Geometry: see drawing. Coordinates: mm, zero at the bounding-box minimum. Round coordinates to 2 decimals unless told otherwise and drop trailing zeros. Write each loop counter-clockwise with the first axis right and the second up, starting at its lowest first coordinate (ties: lowest second). Pieces come first, ordered by that corner, then holes. Notation, with made-up numbers: M 7.5,-30 L 27.5,-30 A30 cw 27.5,-5 Z; hole C 72,-28 d3. An arc over 180 degrees is marked long. Write each question's results on one line, items separated by ' | '. Start each with the question number.
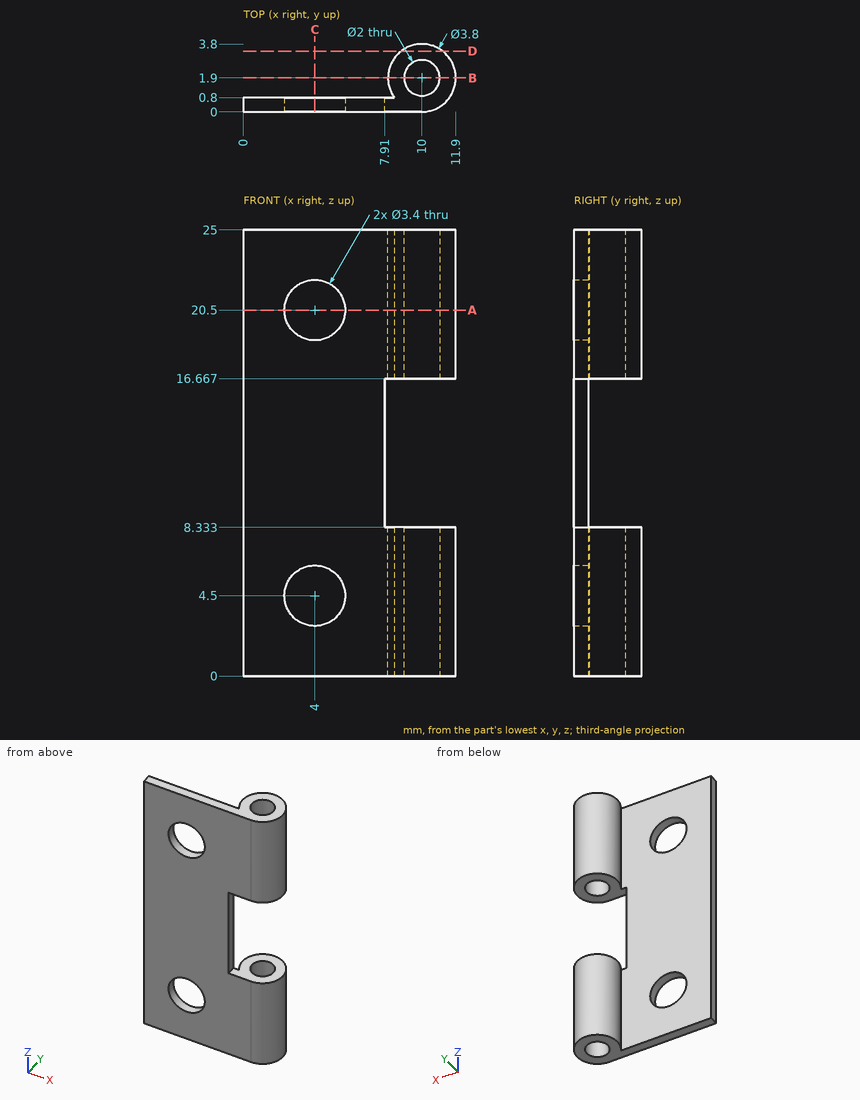
1. Cut plane D-D on y = 3.4. Output: boundary loops of the cut face in (x, z).
2. Cut plane B-B on y = 1.9. Output: boundary loops of the cut face in (x, z).
3. Cut plane A-A on z = 20.5. Output: boundary loops of the cut face in (x, y), and give its area (3 significant figures).
4. Contact query for a flat-ended pin moving along its axis: P1, Ø1.1, axis at x = 9.5, y = 1.5, coming from the -Z side. Output: stop coordinate, or through.
5. Cut plane C-C on x = 4. Output: boundary loops of the cut face in (y, z).
6. Line query: L1, parallel to X at y = 1.85, z = 3.5; L2, parallel to Z at x = 9.75, y = 3.15; L3, parallel to Y at x = 5.25, z = 16. Output: solid intervals per line, ascending. Write a range as from..to.
Answers follow:
1) outline: M 8.83,0 L 11.17,0 L 11.17,8.33 L 8.83,8.33 Z; M 8.83,16.67 L 11.17,16.67 L 11.17,25 L 8.83,25 Z
2) outline: M 8.1,0 L 9,0 L 9,8.33 L 8.1,8.33 Z; M 8.1,16.67 L 9,16.67 L 9,25 L 8.1,25 Z; M 11,0 L 11.9,0 L 11.9,8.33 L 11,8.33 Z; M 11,16.67 L 11.9,16.67 L 11.9,25 L 11,25 Z
3) outline: M 0,0 L 2.3,0 L 2.3,0.8 L 0,0.8 Z; M 5.7,0 L 10,0 A1.9 ccw long 8.45,0.8 L 5.7,0.8 Z; hole C 10,1.9 d2 | area: 12.6 mm2
4) P1: stops at z = 0
5) outline: M 0,0 L 0.8,0 L 0.8,2.8 L 0,2.8 Z; M 0,6.2 L 0.8,6.2 L 0.8,18.8 L 0,18.8 Z; M 0,22.2 L 0.8,22.2 L 0.8,25 L 0,25 Z
6) L1: x = 8.1..9, 11..11.9 | L2: z = 0..8.33, 16.67..25 | L3: y = 0..0.8
